from build123d import *

# Parameters (mm, degrees)
BOSS_EXTRUDE1_DEPTH   = 40
SKETCH2_W             = 52
SKETCH2_H             = 20
CUT_EXTRUDE1_DEPTH    = 56
SKETCH3_R             = 5
CUT_EXTRUDE2_DEPTH    = 56
CHAMFER1_SIZE         = 20
SKETCH4_W             = 30
SKETCH4_H             = 11
BOSS_EXTRUDE2_DEPTH   = 15
SKETCH5_R             = 5
BOSS_EXTRUDE3_DEPTH   = 15
SKETCH6_W             = 45
SKETCH6_H             = 20
BOSS_EXTRUDE4_DEPTH   = 10
CUT_EXTRUDE3_REACH    = 134.714
SKETCH8_W             = 47.061475946
SKETCH8_H             = 40
SKETCH9_W             = 45
SKETCH9_H             = 19
BOSS_EXTRUDE5_DEPTH   = 8
SKETCH11_R            = 2.75
CUT_EXTRUDE4_DEPTH    = 37
SKETCH12_W            = 30
SKETCH12_H            = 100
CUT_EXTRUDE5_DEPTH    = 112
SKETCH13_W            = 0.2
SKETCH13_H            = 62
CUT_EXTRUDE6_DEPTH    = 112
CHAMFER2_SIZE         = 0.5
SKETCH14_W            = 1
SKETCH14_H            = 9.442903458
CUT_EXTRUDE7_DEPTH    = 29
SKETCH15_R            = 2.25
CUT_EXTRUDE8_DEPTH    = 9.5
M4_TAPPED_HOLE1_D     = 3.3
M4_TAPPED_HOLE1_DEPTH = 9.5
M4_TAPPED_HOLE2_D     = 3.3
M4_TAPPED_HOLE2_DEPTH = 9.5
FILLET1_R             = 5


with BuildPart() as part:
    # Sketch1 → Boss-Extrude1 (new body)
    with BuildSketch(Plane(origin=(0, 0, 0), x_dir=(1, 0, 0), z_dir=(0, 1, 0))):
        Polygon((0, 0), (72, 0), (72, 15), (10, 15), (10, 45), (0, 45), align=None)
    extrude(amount=BOSS_EXTRUDE1_DEPTH)

    # Sketch2 → Cut-Extrude1 (cut)
    with BuildSketch(Plane.XY):
        with Locations((26, 10)):
            Rectangle(SKETCH2_W, SKETCH2_H)
    extrude(amount=-CUT_EXTRUDE1_DEPTH, mode=Mode.SUBTRACT)

    # Sketch3 → Cut-Extrude2 (cut)
    with BuildSketch(Plane.XY):
        with Locations((62, 13)):
            Circle(SKETCH3_R)
    extrude(amount=-CUT_EXTRUDE2_DEPTH, mode=Mode.SUBTRACT)

    # Chamfer1
    chamfer1_edges = [part.edges().sort_by_distance(p)[0] for p in [
        (72, 40, -7.5),
    ]]
    chamfer(chamfer1_edges, length=CHAMFER1_SIZE)

    # Sketch4 → Boss-Extrude2 (add)
    with BuildSketch(Plane.XY):
        with Locations((37, 45.5)):
            Rectangle(SKETCH4_W, SKETCH4_H)
    extrude(amount=-BOSS_EXTRUDE2_DEPTH)

    # Sketch5 → Boss-Extrude3 (add)
    with BuildSketch(Plane.XY):
        Polygon((22, 51), (52, 51), (52, 62), (72, 82), (72, 102), (52, 102), (52, 82), (0, 82), (0, 62), (22, 62), align=None)
        with Locations((62, 89)):
            Circle(SKETCH5_R, mode=Mode.SUBTRACT)
    extrude(amount=-BOSS_EXTRUDE3_DEPTH)

    # Sketch6 → Boss-Extrude4 (add)
    with BuildSketch(Plane.ZY):
        with Locations((-22.5, 30)):
            Rectangle(SKETCH6_W, SKETCH6_H)
        with Locations((-22.5, 72)):
            Rectangle(SKETCH6_W, SKETCH6_H)
    extrude(amount=-BOSS_EXTRUDE4_DEPTH)

    # Cut-Extrude3: up to this face of the body (flat: up to its plane)
    cut_extrude3_end = Plane(part.part.faces().sort_by_distance((22, 51, -7.5))[0])
    # Sketch8 → Cut-Extrude3 (cut, up to the picked face)
    with BuildSketch(Plane.ZY, mode=Mode.PRIVATE) as cut_extrude3_sk1:
        with Locations((-21.469262027, 51)):
            Rectangle(SKETCH8_W, SKETCH8_H)
    cut_extrude3_tool1 = split(extrude(cut_extrude3_sk1.sketch, amount=-CUT_EXTRUDE3_REACH, mode=Mode.PRIVATE), bisect_by=cut_extrude3_end, keep=Keep.BOTH, mode=Mode.PRIVATE)
    add(cut_extrude3_tool1.solids().sort_by(Axis((0, 51, -21.469262), (1, 0, 0)))[0], mode=Mode.SUBTRACT)

    # Sketch9 → Boss-Extrude5 (add)
    with BuildSketch(Plane(origin=(10, 0, 0), x_dir=(0, 0, -1), z_dir=(1, 0, 0))):
        with Locations((22.5, 91.5)):
            Rectangle(SKETCH9_W, SKETCH9_H)
        with Locations((22.5, 10.5)):
            Rectangle(SKETCH9_W, SKETCH9_H)
    extrude(amount=-BOSS_EXTRUDE5_DEPTH)

    # Sketch11 → Cut-Extrude4 (cut)
    with BuildSketch(Plane(origin=(10, 0, 0), x_dir=(0, 0, -1), z_dir=(1, 0, 0))):
        with Locations((7.5, 93.5)):
            Circle(SKETCH11_R)
        with Locations(Location((7.5, 8.5, 0), (0, 0, 180))):
            Circle(SKETCH11_R)
    extrude(amount=-CUT_EXTRUDE4_DEPTH, mode=Mode.SUBTRACT)

    # Sketch12 → Cut-Extrude5 (cut)
    with BuildSketch(Plane(origin=(72, 0, 0), x_dir=(0, 0, -1), z_dir=(1, 0, 0))):
        with Locations((30, 51)):
            Rectangle(SKETCH12_W, SKETCH12_H)
    extrude(amount=-CUT_EXTRUDE5_DEPTH, mode=Mode.SUBTRACT)

    # Sketch13 → Cut-Extrude6 (cut)
    with BuildSketch(Plane.XY):
        with Locations((0.1, 51)):
            Rectangle(SKETCH13_W, SKETCH13_H)
    extrude(amount=-CUT_EXTRUDE6_DEPTH, mode=Mode.SUBTRACT)

    # Chamfer2
    chamfer2_edges = [part.edges().sort_by_distance(p)[0] for p in [
        (0.2, 20, -7.5),
        (0.2, 82, -7.5),
    ]]
    chamfer(chamfer2_edges, length=CHAMFER2_SIZE)

    # Sketch14 → Cut-Extrude7 (cut)
    with BuildSketch(Plane.XY):
        with Locations((62, 4.721451729)):
            Rectangle(SKETCH14_W, SKETCH14_H)
        with Locations((62, 97.278548271)):
            Rectangle(SKETCH14_W, SKETCH14_H)
    extrude(amount=-CUT_EXTRUDE7_DEPTH, mode=Mode.SUBTRACT)

    # Sketch15 → Cut-Extrude8 (cut)
    with BuildSketch(Plane(origin=(72, 0, 0), x_dir=(0, 0, -1), z_dir=(1, 0, 0))):
        with Locations((7.5, 97.75)):
            Circle(SKETCH15_R)
        with Locations((7.5, 4.25)):
            Circle(SKETCH15_R)
    extrude(amount=-CUT_EXTRUDE8_DEPTH, mode=Mode.SUBTRACT)

    # M4 Tapped Hole1
    with Locations(Plane(origin=(61.5, 97.75, -7.5), x_dir=(0, 0, 1), z_dir=(1, 0, 0))):
        with Locations((0, 0)):
            Hole(M4_TAPPED_HOLE1_D / 2, depth=M4_TAPPED_HOLE1_DEPTH)

    # M4 Tapped Hole2
    with Locations(Plane(origin=(61.5, 4.25, -7.5), x_dir=(0, 0, 1), z_dir=(1, 0, 0))):
        with Locations((0, 0)):
            Hole(M4_TAPPED_HOLE2_D / 2, depth=M4_TAPPED_HOLE2_DEPTH)

    # Fillet1
    fillet1_edges = [part.edges().sort_by_distance(p)[0] for p in [
        (72, 20, -7.5),
        (72, 82, -7.5),
        (52, 62, -7.5),
        (52, 40, -7.5),
        (52, 82, -7.5),
        (10, 82, -7.5),
        (22, 71, -7.5),
        (22, 31, -7.5),
        (10, 20, -7.5),
        (52, 20, -7.5),
    ]]
    fillet(fillet1_edges, radius=FILLET1_R)


solid = part.part
CAD build for the part. Positions are in the model's coordinates, mm. A direction names the side the tool comes from. Round coordinates to 2 decimals unless told otherwise and drop trailing zeros. Loops run counter-clockwise (first coordinate to the right, second up) from the corner with the lowest first, then second, coordinate; pieces in that order, holes last.
(1) Two-plate mould, pull along X, no slides. Class faces 1 (the cylindrical face through (71.63, 82.18, -7.6)), 2 (the flat face through (31, 20, -7)), 3 (the flat face through (0.2, 76, -7)): +X half, -X half, draft (parallel to the pull), parting line (faces both ways), or undercut.
(2) Wall check: line 1 along Y through (x, z) = (5.25, -7.5); line 2 along Y through (x, z) = (54.5, -7.5); line 3 along X through (y, z) = (7.5, -6.25). Give the ranges that are in metal, low to high.
(3) Which spindle directions (+Z, -Z, +X, -X, +Y, -Y) get a long thin tool onto all of the face, cutting with end or side? Do faces 4 (the cylindrical face through (6.06, 91.06, -8.77)), 5 (the flat face through (6, 1, -7)), 6 (the cylindrical face through (52.39, 61.87, -7.6)), 7 (the cylindrical face through (20, 32, -8)). Say none if no direction does.
(4) Cut at C-C (x = 43). Give the cut face in (y, z).
(5) Drop flat-ended pins along their axis: pin 1 (4 mm diameter, centred on y = 97.75, z = -7.5, fed in from -X); pin 2 (7.5 mm diameter, centred on y = 56, z = -9, fed in from -X); pin 3 (1 mm diameter, centred on x = 26, z = -8, fed in from -Y); pin 4 (8 mm diameter, centred on x = 62, y = 89, fed in from -Z). Give the stop position or say it passes through.
(6) Cut at B-B (z = -7.5). State how many separate pieces and enclosed holes the cut face has, plus the area to 3 significant figures.
(7) Cut at A-A (y = 97.75). Give the cut face in (x, z), plus the area to 3 significant figures.
Findings below:
1. face 1: +X half
1. face 2: undercut
1. face 3: -X half
2. line 1: y = 1 to 5.75, 11.25 to 31, 71 to 90.75, 96.25 to 101
2. line 2: y = 0 to 2.6, 5.9 to 37.5, 64.5 to 96.1, 99.4 to 102
2. line 3: x = 52 to 61.5, 62.5 to 72
3. face 4: -X
3. face 5: +Z, -Z, -X, -Y
3. face 6: +Z, -Z, +X
3. face 7: +Z, -Z, -X
4. outline: (20, -15) - (82, -15) - (82, 0) - (20, 0) - close
5. pin 1: stops at x = 2
5. pin 2: stops at x = 22
5. pin 3: stops at y = 20
5. pin 4: passes through
6. separate pieces: 7
6. enclosed holes: 0
6. area: 3,470 mm2
7. outline: (2, -15) - (10, -15) - (10, 0) - (2, 0) - close; (52, -15) - (61.5, -15) - (61.5, -9.15) - (52, -9.15) - close; (52, -5.85) - (61.5, -5.85) - (61.5, 0) - (52, 0) - close; (62.5, -15) - (72, -15) - (72, -9.75) - (62.5, -9.75) - close; (62.5, -5.25) - (72, -5.25) - (72, 0) - (62.5, 0) - close
7. area: 331 mm2
